The listing builds one solid part. Answer for the finished solid, in the listing's coordinates (mm). A direction names the side the tool comes from. Give positions to 0.01 mm unless a question says otherwise; leave off trailing zeros. Order: outer loops, then holes, each group sorted by start corner. A loop starts at its lowest first (then second) coordinate and runs counter-clockwise, first axis right, second up. Notation, with made-up numbers: (39, -14.5) - (78, -14.5) arc R11 cw to (78, 6.5) - close; hole circle Ø11 at (18.5, 87.5). An arc over 180 degrees is marked (long way). Answer in a Markdown table with one row per item. Add a question column.
```python
from build123d import *

# Parameters (mm, degrees)
BOSS_EXTRUDE1_DEPTH = 310
BOSS_EXTRUDE2_START = -26
SKETCH2_R           = 5
BOSS_EXTRUDE2_DEPTH = 55


with BuildPart() as part:
    # Sketch1 → Boss-Extrude1 (new, symmetric)
    with BuildSketch(Plane.XY):
        Polygon((0, 0), (7.5, 12.990381057), (0, 25.980762114), (0, 78.421161675), (-7.267949192, 91.009618943), (-0.200961894, 103.25), (-1.5, 104), (-9, 91.009618943), (-1.5, 78.019237886), (-1.5, 25.578838325), (5.767949192, 12.990381057), (-1.299038106, 0.75), align=None)
    extrude(amount=BOSS_EXTRUDE1_DEPTH, both=True)

    # Sketch2 → Boss-Extrude2 (add)
    with BuildSketch(Plane.XY.offset(310).offset(BOSS_EXTRUDE2_START)):
        with Locations((-0.75, 56.5)):
            Circle(SKETCH2_R)
    boss_extrude2 = extrude(amount=BOSS_EXTRUDE2_DEPTH)

    # Mirror1: Boss-Extrude2 across plane
    add(boss_extrude2.mirror(Plane.XY))


solid = part.part
```
(1) Find section B-B, the plane y = 33.5. Write down the section's boundary in (x, z), plus the area to 3 significant figures.
(2) For faces 1 (the face through (2.284, 6.956, 4.34)), 2 (the face through (-3.784, 97.044, 4.34)), 3 (the face through (-5.198, 97.596, 4.34)), determine the directions among +Z, -Z, +X, -X, +Y, -Y from which every point of the face is accessible in a straight line to the end or side of a thin tool.
(3) Find section A-A, the plane z = -296.5. Write down the section's boundary in (x, y), plus the area to 3 significant figures.
(4) Each of these flat-tipped pins is pushed along its axis until it touches: P1, Ø7, axis at x = 3.5, y = 26.5, coming from the +Z side; P2, Ø2.5, axis at x = 2.5, y = 33.5, coming from the -Z side; P3, Ø5, axis at y = 93, z = -246.5, coming from the +X side; P4, Ø2, axis at x = 0, z = -225.5, coming from the +Y side. Where does it stop, or does it pass through?
(5) Straight lines are drawn through the part: line 1 (Y direction, x = -0.5, z = 110); line 2 (X direction, y = 62.5, z = -207); line 3 (Y direction, x = -2, z = -151). For each, find the intervals that lie inside material, in ascending order.
(6) The mould has two halves that part along Z. Classify faces 4 (the face through (0, 52, 4)), 5 (the face through (2.083, 19.373, 4.34)), 6 (the face through (-1.5, 52, 4)): +Z half, -Z half, draft (parallel to the pull), parting line (faces both ways), or undercut.
(7) Find section C-C, the plane z = -65. Write down the section's boundary in (x, y), plus the area to 3 significant figures.
Answer key:
| question | item | result |
|---|---|---|
| 1 | outline | (-1.5, -310) - (0, -310) - (0, 310) - (-1.5, 310) - close |
| 1 | area | 930 mm² |
| 2 | face 1 | +Z, -Z, -X |
| 2 | face 2 | +Z, -Z, +X |
| 2 | face 3 | +Z, -Z, -X, +Y |
| 3 | outline | (-9, 91.01) - (-1.5, 78.02) - (-1.5, 61.44) arc R5 ccw to (-1.5, 51.56) - (-1.5, 25.58) - (5.77, 12.99) - (-1.3, 0.75) - (0, 0) - (7.5, 12.99) - (0, 25.98) - (0, 51.56) arc R5 ccw to (0, 61.44) - (0, 78.42) - (-7.27, 91.01) - (-0.2, 103.25) - (-1.5, 104) - close |
| 3 | area | 230 mm² |
| 4 | P1 | z = 310 |
| 4 | P2 | through |
| 4 | P3 | x = -4.68 |
| 4 | P4 | y = 103.71 |
| 5 | line 1 | 0.29 to 2.13, 23.85 to 79.29, 102.73 to 103.42 |
| 5 | line 2 | -1.5 to 0 |
| 5 | line 3 | 78.89 to 81.89, 100.13 to 103.13 |
| 6 | face 4 | undercut |
| 6 | face 5 | draft |
| 6 | face 6 | undercut |
| 7 | outline | (-9, 91.01) - (-1.5, 78.02) - (-1.5, 25.58) - (5.77, 12.99) - (-1.3, 0.75) - (0, 0) - (7.5, 12.99) - (0, 25.98) - (0, 78.42) - (-7.27, 91.01) - (-0.2, 103.25) - (-1.5, 104) - close |
| 7 | area | 167 mm² |
